Can you work these out from the model? Positions are in its coordinate system, mm. Face numbers are marked on the shaded views. Give positions to 0.01 mm unless a question says otherwise; leave off trailing zeros. Loops run counter-clockwise (first coordinate to the right, second up) from the corner with the lowest first, then second, coordinate; pieces in that order, holes last. Notation, with made-up numbers: M 37,-19 L 48,-19 A16 cw 48,-2 Z; hole C 66,-10.5 d4. An arc over 180 degrees is marked long. Answer as a JSON object with one key per item and string values.
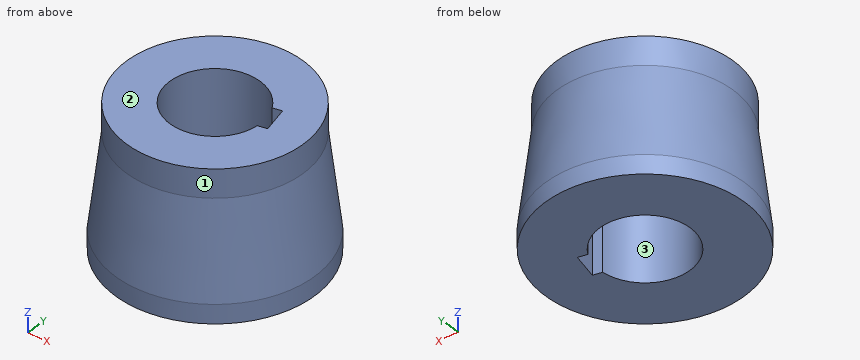
```python
from build123d import *

# Parameters (mm, degrees)
CUT_EXTRUDE1_DEPTH = 647.654791602
SKETCH3_W          = 24
SKETCH3_H          = 75


with BuildPart() as part:
    # Sketch1 → Revolve1 (revolve)
    with BuildSketch(Plane.XZ.offset(-234.743963655), mode=Mode.PRIVATE) as revolve1_sk:
        Polygon((568.230642584, -1074.998443067), (521.230642584, -1074.998443067), (521.230642584, -1149.998443067), (574.230642584, -1149.998443067), (574.230642584, -1139.998443067), (568.230642584, -1089.998443067), align=None)
    revolve(revolve1_sk.sketch.rotate(Axis((521.230642584, 234.743963655, -1074.998443067), (0, 0, -1)), 270), axis=Axis((521.230642584, 234.743963655, -1074.998443067), (0, 0, -1)))

    # Sketch2 → Cut-Extrude1 (cut, through all)
    with BuildSketch(Plane.XY.offset(-1074.998443067)):
        with BuildLine():
            Line((549.898349026, 234.692901362), (546.50406086, 248.275198952))
            Line((546.50406086, 248.275198952), (541.805052122, 247.10089176))
            ThreePointArc((541.805052122, 247.10089176), (544.514581311, 240.562743369), (545.199340288, 233.518594169))
            Line((545.199340288, 233.518594169), (549.898349026, 234.692901362))
        make_face()
    extrude(amount=-CUT_EXTRUDE1_DEPTH, mode=Mode.SUBTRACT)

    # Sketch3 → Cut-Revolve1 (revolve, cut)
    with BuildSketch(Plane.XZ.offset(-234.743963655)):
        with Locations((533.230642584, -1112.498443067)):
            Rectangle(SKETCH3_W, SKETCH3_H)
    revolve(axis=Axis((521.230642584, 234.743963655, -1074.998443067), (0, 0, -1)), mode=Mode.SUBTRACT)


solid = part.part
```
1) Suppose I cut it at A-A, the plane z = -1107. Write out the boundary of the cut face in (x, y).
Answer list:
{"outline": "C 521.23,234.74 d98.08; hole M 541.81,247.1 A24 ccw long 545.2,233.52 L 549.9,234.69 L 546.5,248.28 Z"}
2) Please list where these lines run through material, in increasing order: line 1 along Y through (x, z) = (546, -1107); line 2 along X through (y, z) = (246.5, -1082.5); line 3 along Y through (x, z) = (534, -1137). Write a range as from..to.
Answer list:
{"line 1": "192.42..233.72, 248.15..277.07", "line 2": "475.72..500.31, 546.95..566.74", "line 3": "183.68..214.42, 255.06..285.81"}
3) Will these pins go through, and if not, where does the flat tip stop? pin 1 Ø12 at (y, z) = (273, -1106) entering from +X; pin 2 Ø10 at (y, z) = (215, -1122) entering from -X; pin 3 Ø4 at (x, z) = (494.5, -1100.5) entering from -Y.
Answer list:
{"pin 1": "x = 558.1", "pin 2": "x = 472.45", "pin 3": "y = 193.27"}
4) If we mould it in two halves opening along X, with no side actions, what happens to the marked faces 1, 2 and 3? For each: +X half, -X half, draft (parallel to the pull), parting line (faces both ways), or undercut.
Answer list:
{"face 1": "parting line", "face 2": "draft", "face 3": "undercut"}
5) Suppose I cut it at B-B, the plane z = -1144.5. Write out the boundary of the cut face in (x, y).
Answer list:
{"outline": "C 521.23,234.74 d106; hole M 541.81,247.1 A24 ccw long 545.2,233.52 L 549.9,234.69 L 546.5,248.28 Z"}
